Geometry check sheet. Reference: drawing and pictorial views, mm from the part's lowest x, y, z. A direction names the side the tool comes from. Give positions to 0.01 mm unless a question says otherwise; leave off trailing zeros. Loops run counter-clockwise (first coordinate to the right, second up) from the corner with the lowest first, then second, coordinate; pieces in that order, holes last. Notation, with made-up numbers: (19, 73) - (78, 73) arc R25 cw to (78, 109) - close; hole circle Ø7 at (8, 44). An arc over 180 degrees is marked (long way). Put each result on its own line as item: value. Start each with the question number.
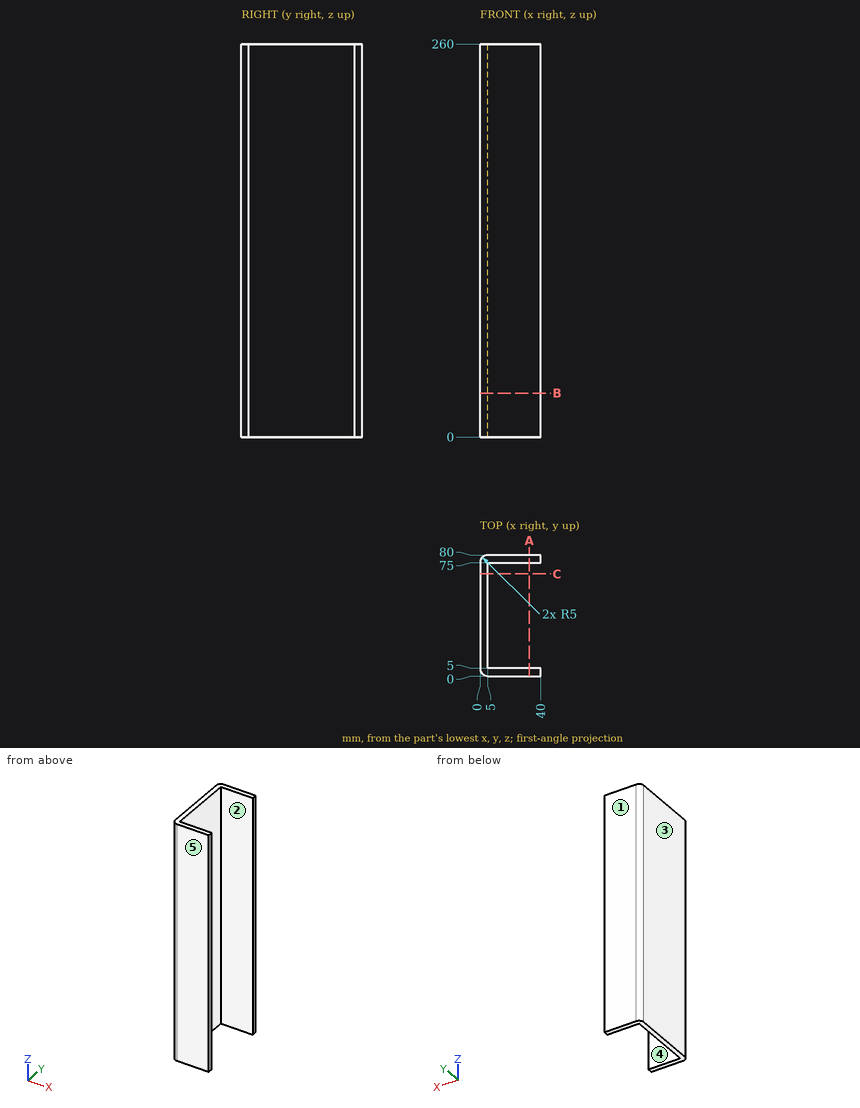
1) Section check B-B, the plane z = 29. Enter the section's corners in (x, y), plus the area to 3 significant figures.
2) Set-up check for the marked faces 1 and 2: record each of +Z, -Z, +X, -X, +Y, -Y from which the full face is reachable in a straight line by a thin tool's end or side.
3) Section check C-C, the plane y = 67.5. Enter the section's corners in (x, z).
4) Depth check by flat-ended pin: P1, Ø12, axis at x = 6, z = 49, coming from the -Y side; P2, Ø21, axis at y = 40.5, z = 163.5, coming from the +X side. Enter the tip coordinate at first touch or a pass-through.
5) Scan lines: line 1 along Y through (x, z) = (22, 172); line 2 along X through (y, z) = (14, 41.5); line 3 along X through (y, z) = (4, 91). Record each from-to range of solid material in increasing order. Write a range as from..to.
6) Draft check along Y on the marked faces 3, 4 and 5. Enter one of: pulls with the +Y half, pulls with the -Y half, needs draft (parallel to the pull), parting line crosses it, or undercut.
7) Section check A-A, the plane x = 32.5. Enter the section's corners in (y, z), plus the area to 3 significant figures.
Results are:
1. outline: (0, 5) arc R5 ccw to (5, 0) - (40, 0) - (40, 5) - (5, 5) - (5, 75) - (40, 75) - (40, 80) - (5, 80) arc R5 ccw to (0, 75) - close
1. area: 739 mm2
2. face 1: +Z, -Z, +X, -X, +Y
2. face 2: +Z, -Z, +X
3. outline: (0, 0) - (5, 0) - (5, 260) - (0, 260) - close
4. P1: stops at y = 0
4. P2: stops at x = 5
5. line 1: y = 0..5, 75..80
5. line 2: x = 0..5
5. line 3: x = 0.1..40
6. face 3: needs draft
6. face 4: undercut
6. face 5: pulls with the -Y half
7. outline: (0, 0) - (5, 0) - (5, 260) - (0, 260) - close; (75, 0) - (80, 0) - (80, 260) - (75, 260) - close
7. area: 2,600 mm2
